Work out the finished part from the listing and answer in its coordinate system (mm). Face numbers are marked on the shaded views. Coordinates: 2 decimals unless noted, no trailing zeros. Order: outer loops, then holes, each group sorted by start corner. A loop starts at its lowest first (then second) coordinate and runs counter-clockwise, first axis right, second up. Notation, with made-up numbers: (49.5, -6) - (84.5, -6) arc R16 ccw to (84.5, 4) - close; hole circle Ø9 at (-20.5, 52). An arc over 180 degrees is marked (long way). Answer as a JSON object with one key per item and string values. Group by question number.
1) Section A-A (z = -20) is taken. Give the vertices of the cut face in (x, y).
2) Section D-D (y = -6.5) is taken. Give the vertices of the cut face in (x, z), plus the area to 3 significant figures.
3) Find the intervals of material crossed by line 1 along Y through (x, z) = (1, 14); line 2 along Z through (x, y) = (6.5, -0.5); line 3 along X through (y, z) = (8, -8), in increasing order.
4) Section C-C (z = 18) is taken. Give the vertices of the cut face in (x, y).
5) The mould has two halves that part along Z. Classify the marked faces 1, 2 and 3: released by +Z, released by -Z, zero draft, split by the parting line, or undercut.
6) Section B-B (y = 0) is taken. Give the vertices of the cut face in (x, z), plus the area to 3 significant figures.
7) Each of these flat-tipped pins is pushed along its axis until it touches: P1, Ø1, axis at y = 2, z = 13.5, coming from the -X side; P2, Ø0.8, axis at x = 0.5, z = 3, coming from the +Y side; P3, Ø3.5, axis at y = -8, z = 8.5, coming from the -X side; P4, Ø1.3, axis at y = -3.5, z = -0.5, coming from the -X side. Where does it stop, or does it pass through?
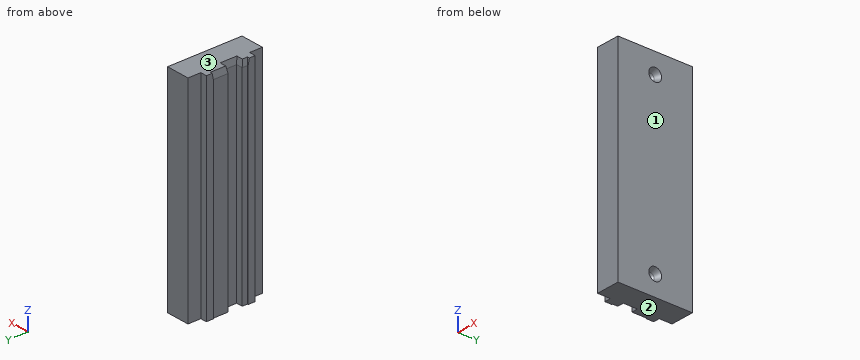
from build123d import *
from OCP.BRepFilletAPI import BRepFilletAPI_MakeChamfer

# Parameters (mm, degrees)
SKETCH1_W           = 49.4
SKETCH1_H           = 17.4
BOSS_EXTRUDE1_DEPTH = 7
SKETCH2_W           = 49.4
SKETCH2_H           = 8.1
CUT_EXTRUDE1_DEPTH  = 0.2
SKETCH3_W           = 49.4
SKETCH3_H           = 3.3
CUT_EXTRUDE2_DEPTH  = 1.7
SKETCH5_W           = 49.4
SKETCH5_H           = 3
CUT_EXTRUDE3_DEPTH  = 1.5
CHAMFER1_SIZE       = 1.5
CHAMFER1_SIZE2      = 0.3
CHAMFER2_SIZE       = 0.3
CHAMFER2_SIZE2      = 1.5


with BuildPart() as part:
    # Sketch1 → Boss-Extrude1 (new body)
    with BuildSketch(Plane(origin=(0, 0, 0), x_dir=(0, 0, -1), z_dir=(1, 0, 0))):
        Rectangle(SKETCH1_W, SKETCH1_H)
    extrude(amount=BOSS_EXTRUDE1_DEPTH)

    # Sketch2 → Cut-Extrude1 (cut)
    with BuildSketch(Plane.ZY):
        Rectangle(SKETCH2_W, SKETCH2_H)
    extrude(amount=-CUT_EXTRUDE1_DEPTH, mode=Mode.SUBTRACT)

    # Sketch3 → Cut-Extrude2 (cut)
    with BuildSketch(Plane.ZY):
        with Locations((0, -1.2)):
            Rectangle(SKETCH3_W, SKETCH3_H)
    extrude(amount=-CUT_EXTRUDE2_DEPTH, mode=Mode.SUBTRACT)

    # Sketch4 → Cut-Revolve1 (revolve, cut)
    with BuildSketch(Plane(origin=(0, 0, 0), x_dir=(1, 0, 0), z_dir=(0, 1, 0))):
        with BuildLine():
            Line((5.617316568, 20.923879533), (7, 21.496605763))
            Line((7, 21.496605763), (7, 20))
            Line((7, 20), (5, 20))
            ThreePointArc((5, 20), (5.168530388, 20.555570233), (5.617316568, 20.923879533))
        make_face()
    cut_revolve1 = revolve(axis=Axis((9.957130438, 0, -20), (1, 0, 0)), mode=Mode.SUBTRACT)

    # Mirror1: Cut-Revolve1 across plane
    add(cut_revolve1.mirror(Plane.XY), mode=Mode.SUBTRACT)

    # Sketch5 → Cut-Extrude3 (cut)
    with BuildSketch(Plane.ZY):
        with Locations((0, 7.2)):
            Rectangle(SKETCH5_W, SKETCH5_H)
        with Locations((0, -7.2)):
            Rectangle(SKETCH5_W, SKETCH5_H)
    extrude(amount=-CUT_EXTRUDE3_DEPTH, mode=Mode.SUBTRACT)

    # Chamfer1: one chamfer whose edges measure the first distance from different faces: ONE call of the kernel's chamfer builder (chamfer() names one face for all edges)
    chamfer1_edges_1 = [part.edges().sort_by_distance(p)[0] for p in [
        (0.2, -3.45, 24.7),
    ]]
    chamfer1_side_1 = [part.faces().sort_by_distance(p)[0] for p in [
        (0.2, -3.45, 0),
    ]]
    chamfer1_edges_2 = [part.edges().sort_by_distance(p)[0] for p in [
        (0.1, -4.05, 24.7),
    ]]
    chamfer1_side_2 = [part.faces().sort_by_distance(p)[0] for p in [
        (0.1, -4.05, 0),
    ]]
    chamfer1_edges_3 = [part.edges().sort_by_distance(p)[0] for p in [
        (0.95, -2.85, 24.7),
    ]]
    chamfer1_side_3 = [part.faces().sort_by_distance(p)[0] for p in [
        (0.95, -2.85, 0),
    ]]
    chamfer1 = BRepFilletAPI_MakeChamfer(part.part.solid().wrapped)
    for e in chamfer1_edges_1:
        chamfer1.Add(CHAMFER1_SIZE, CHAMFER1_SIZE2, e.wrapped, chamfer1_side_1[0].wrapped)  # the first distance lies on this face
    for e in chamfer1_edges_2:
        chamfer1.Add(CHAMFER1_SIZE, CHAMFER1_SIZE2, e.wrapped, chamfer1_side_2[0].wrapped)  # the first distance lies on this face
    for e in chamfer1_edges_3:
        chamfer1.Add(CHAMFER1_SIZE, CHAMFER1_SIZE2, e.wrapped, chamfer1_side_3[0].wrapped)  # the first distance lies on this face
    add(Compound.cast(chamfer1.Shape()), mode=Mode.REPLACE)

    # Chamfer2
    chamfer2_edges = [part.edges().sort_by_distance(p)[0] for p in [
        (1.7, -1.35, 24.7),
        (0.1, 4.05, 24.7),
        (0.2, 2.25, 24.7),
        (0.95, 0.45, 24.7),
    ]]
    chamfer2_side = [part.faces().sort_by_distance(p)[0] for p in [
        (3.930580866, 0.084396355, 24.7),
    ]]
    chamfer(chamfer2_edges, length=CHAMFER2_SIZE, length2=CHAMFER2_SIZE2, reference=chamfer2_side[0])


solid = part.part
Report:
{
 "1": {"outline": "(0, -5.7) - (1.5, -5.7) - (1.5, -8.7) - (7, -8.7) - (7, -1.5) - (5.62, -0.92) arc R1 cw to (5.62, 0.92) - (7, 1.5) - (7, 8.7) - (1.5, 8.7) - (1.5, 5.7) - (0, 5.7) - (0, 4.05) - (0.2, 4.05) - (0.2, 0.45) - (1.7, 0.45) - (1.7, -2.85) - (0.2, -2.85) - (0.2, -4.05) - (0, -4.05) - close"},
 "2": {"outline": "(1.5, -24.7) - (7, -24.7) - (7, 24.7) - (1.5, 24.7) - close", "area": "272 mm²"},
 "3": {"line 1": "y = -5.7 to -2.85, 0.45 to 5.7", "line 2": "z = -24.7 to -21.19, -18.81 to 18.81, 21.19 to 24.7", "line 3": "x = 1.5 to 7"},
 "4": {"outline": "(0, -5.7) - (1.5, -5.7) - (1.5, -8.7) - (7, -8.7) - (7, 8.7) - (1.5, 8.7) - (1.5, 5.7) - (0, 5.7) - (0, 4.05) - (0.2, 4.05) - (0.2, 0.45) - (1.7, 0.45) - (1.7, -2.85) - (0.2, -2.85) - (0.2, -4.05) - (0, -4.05) - close"},
 "5": {"face 1": "zero draft", "face 2": "released by -Z", "face 3": "released by +Z"},
 "6": {"outline": "(1.7, -24.7) - (7, -24.7) - (7, -21.5) - (5.62, -20.92) arc R1 cw to (5.62, -19.08) - (7, -18.5) - (7, 18.5) - (5.62, 19.08) arc R1 cw to (5.62, 20.92) - (7, 21.5) - (7, 24.7) - (2, 24.7) - (1.7, 23.2) - close", "area": "253 mm²"},
 "7": {"P1": "stops at x = 0.2", "P2": "stops at y = 5.7", "P3": "stops at x = 1.5", "P4": "stops at x = 0"}
}
